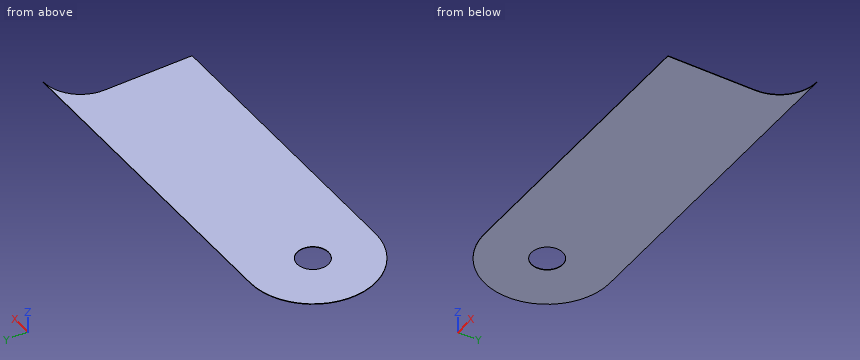
from build123d import *

# Parameters (mm, degrees)
SKETCH1_R           = 63.5
BOSS_EXTRUDE1_DEPTH = 1


with BuildPart() as part:
    # Sketch1 → Boss-Extrude1 (new, symmetric)
    with BuildSketch(Plane.XY):
        with BuildLine():
            Line((0, 254), (1320.8, 254))
            ThreePointArc((1320.8, 254), (1213.036926547, 209.363073453), (1168.4, 101.6))
            Line((1168.4, 101.6), (1168.4, -254))
            Line((1168.4, -254), (0, -254))
            ThreePointArc((0, -254), (-254, 0), (0, 254))
        make_face()
        Circle(SKETCH1_R, mode=Mode.SUBTRACT)
    extrude(amount=BOSS_EXTRUDE1_DEPTH, both=True)


solid = part.part
Design review of the part built by this model. Coordinates are the model's own, in mm. Give positions to 0.01 mm unless a question says otherwise; leave off trailing zeros. Loops run counter-clockwise (first coordinate to the right, second up) from the corner with the lowest first, then second, coordinate; pieces in that order, holes last. Notation, with made-up numbers: (66, 40) -> (72, 40) arc R18 ccw to (72, 63) -> close; hole circle Ø8 at (-2.75, 13.5). An arc over 180 degrees is marked (long way). One line per question, with ' | ' between items. Start each with the question number.
(1) For line 1 (Y direction, x = 0, z = 0.2); line 2 (X direction, y = -57.5, z = 0.35); line 3 (X direction, y = -29, z = -0.85), list the stretches that pass through material, from the lowest coordinate up.
(2) We need section C-C (x = -100). State the section outline as (y, z) points, and give its area (3 significant figures).
(3) Insertion check: P1, Ø1, axis at x = -39, z = 0, coming from the +Y side. The pin has a flat end and moves straight along its axis. Give the tip position at first contact, or say it passes through.
(4) We need section A-A (y = 0). State the section outline as (x, z) points.
(5) We need section B-B (z = -0.6). State the section outline as (x, y) points, and give its area (3 significant figures).
(6) We need section D-D (y = 183.5). State the section outline as (x, z) points, and give its area (3 significant figures).
The answers:
1) line 1: y = -254 to -63.5, 63.5 to 254 | line 2: x = -247.41 to -26.94, 26.94 to 1168.4 | line 3: x = -252.34 to -56.49, 56.49 to 1168.4
2) outline: (-233.49, -1) -> (233.49, -1) -> (233.49, 1) -> (-233.49, 1) -> close | area: 934 mm^2
3) P1: stops at y = 251.07
4) outline: (-254, -1) -> (-63.5, -1) -> (-63.5, 1) -> (-254, 1) -> close; (63.5, -1) -> (1168.4, -1) -> (1168.4, 1) -> (63.5, 1) -> close
5) outline: (0, -254) -> (1168.4, -254) -> (1168.4, 101.6) arc R152.4 cw to (1320.8, 254) -> (0, 254) arc R254 ccw to start; hole circle Ø127 at (0, 0) | area: 687,000 mm^2
6) outline: (-175.62, -1) -> (1192.28, -1) -> (1192.28, 1) -> (-175.62, 1) -> close | area: 2,740 mm^2
